The drawing under review shows one solid part. Ordinate dimensions are in mm from its lowest x, y, z. Coordinates: 2 decimals unless noted, no trailing zeros. Loops run counter-clockwise (first coordinate to the right, second up) from the corner with the lowest first, then second, coordinate; pieces in that order, holes last. Notation, with made-up numbers: M 35.25,71 L 61.25,71 A22 cw 61.25,91 Z; hole C -26.5,-30 d9. An arc over 180 degrees is marked long. Answer as a JSON object with one key per item and string values. Group by question number.
1. Consider section D-D (x = 20). State the section outline as (y, z) points.
2. To check wall thickness, follow probe 1 along Y at (x, z) = (20, 4.75); probe 2 along X at (y, z) = (215, 5.5); probe 3 along Y at (x, z) = (51.5, 3.25). State the ranges of each line that lie inside material, in increasing order.
3. Consider section A-A (y = 15). State the section outline as (x, z) points, then the cut area to 3 significant figures.
4. Consider section C-C (z = 1.75). State the section outline as (x, y) points.
5. Consider section B-B (x = 30). State the section outline as (y, z) points, then the cut area to 3 significant figures.
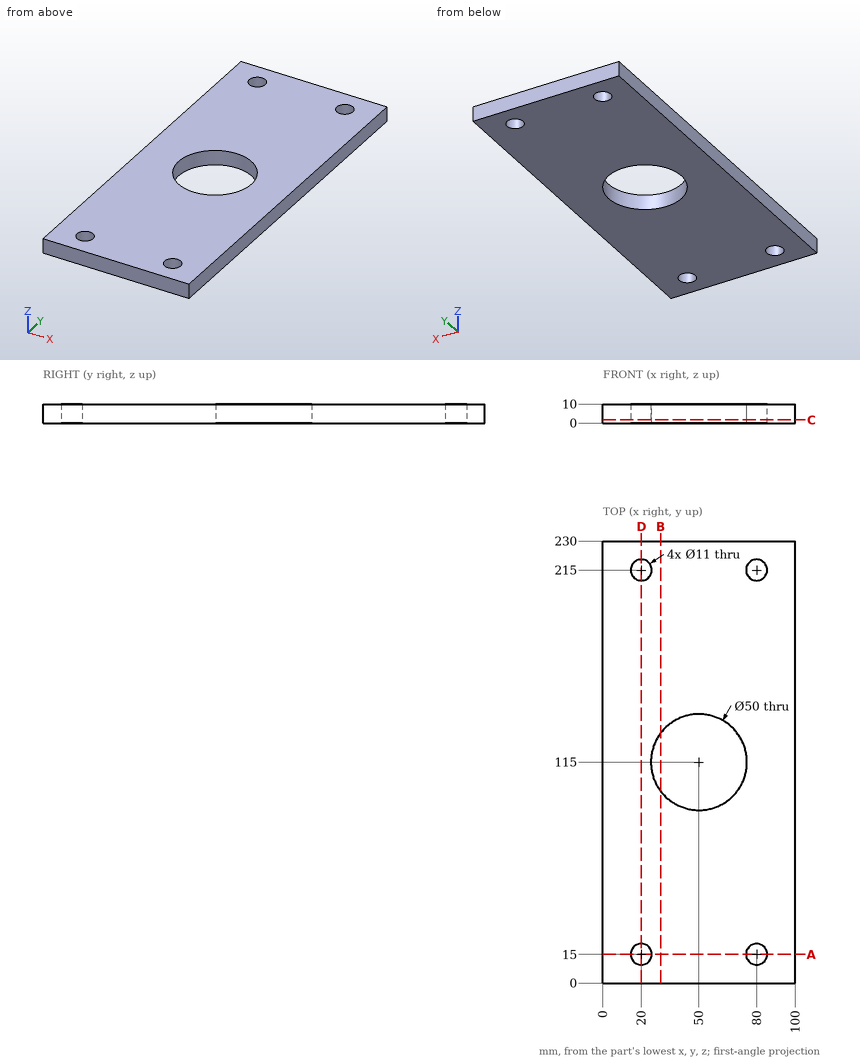
Findings below:
{
 "1": {"outline": "M 0,0 L 9.5,0 L 9.5,10 L 0,10 Z; M 20.5,0 L 209.5,0 L 209.5,10 L 20.5,10 Z; M 220.5,0 L 230,0 L 230,10 L 220.5,10 Z"},
 "2": {"probe 1": "y = 0 to 9.5, 20.5 to 209.5, 220.5 to 230", "probe 2": "x = 0 to 14.5, 25.5 to 74.5, 85.5 to 100", "probe 3": "y = 0 to 90.05, 139.95 to 230"},
 "3": {"outline": "M 0,0 L 14.5,0 L 14.5,10 L 0,10 Z; M 25.5,0 L 74.5,0 L 74.5,10 L 25.5,10 Z; M 85.5,0 L 100,0 L 100,10 L 85.5,10 Z", "area": "780 mm^2"},
 "4": {"outline": "M 0,0 L 100,0 L 100,230 L 0,230 Z; hole C 20,15 d11; hole C 20,215 d11; hole C 50,115 d50; hole C 80,15 d11; hole C 80,215 d11"},
 "5": {"outline": "M 0,0 L 100,0 L 100,10 L 0,10 Z; M 130,0 L 230,0 L 230,10 L 130,10 Z", "area": "2,000 mm^2"}
}
